Geometry: final body of the model. Coordinates: model frame, mm. Round coordinates to 2 decimals unless told otherwise and drop trailing zeros. Loops run counter-clockwise (first coordinate to the right, second up) from the corner with the lowest first, then second, coordinate; pieces in that order, holes last. Notation, with made-up numbers: (12, -37.75) - (25, -37.75) arc R14 cw to (25, -10.75) - close; hole circle Ø7 at (42.5, -25). An arc over 180 degrees is marked (long way). Answer in a Markdown table with one row per item. Add a question column.
from build123d import *

# Parameters (mm, degrees)
EXTRUDE_1_DEPTH     = 6.8
SKETCH_5_R          = 4
CUT_EXTRUDE_1_DEPTH = 13.03425666


with BuildPart() as part:
    # 草图1 → 凸台-拉伸1 (new body)
    with BuildSketch(Plane.XY):
        Polygon((0, 7.505553499), (-6.5, 3.75277675), (-6.5, -3.75277675), (0, -7.505553499), (6.5, -3.75277675), (6.5, 3.75277675), align=None)
    extrude(amount=EXTRUDE_1_DEPTH)

    # 草图4 → 切除-旋转1 (revolve, cut)
    with BuildSketch(Plane(origin=(0, 0, 0), x_dir=(0, 0, -1), z_dir=(1, 0, 0)), mode=Mode.PRIVATE) as cut_revolve_1_sk:
        Polygon((-6.8, -5.85), (-6.197427805, -7.505553499), (-6.8, -7.505553499), align=None)
    cut_revolve_1 = revolve(cut_revolve_1_sk.sketch.rotate(Axis((0, 0, 6.8), (0, 0, -1)), 119.999999984), axis=Axis((0, 0, 6.8), (0, 0, -1)), mode=Mode.SUBTRACT)

    # 镜向1: 切除-旋转1 across plane
    add(cut_revolve_1.mirror(Plane.XY.offset(3.4)), mode=Mode.SUBTRACT)

    # 草图5 → 切除-拉伸1 (cut, through all)
    with BuildSketch(Plane.XY.offset(6.8)):
        Circle(SKETCH_5_R)
    extrude(amount=-CUT_EXTRUDE_1_DEPTH, mode=Mode.SUBTRACT)


solid = part.part
1) Section B-B, the plane y = 0. Return the cut outline in (x, z).
2) Contact query for flat-ended pins moving along their axis: pin 1 Ø1.5 at (x, z) = (3, 2.5) entering from +Y; pin 2 Ø2 at (y, z) = (-5, 5) entering from +X; pin 3 Ø6.5 at (x, y) = (0, 0) entering from +Z. Output: stop coordinate, or through.
3) Pull-direction query (X, two-part tool) for faces 1 (the cylindrical face through (-0.867, -3.905, 3.448)), 2 (the flat face through (-3.2, 5.66, 3.36)), 3 (the flat face through (6.5, 0, 3)), 4 (the flat face through (3, -4, 6.8)); classes: pulls with the +X half, pulls with the -X half, needs draft (parallel to the pull), parting line crosses it, or undercut.
4) Material intervals for line 1 along Y through (x, z) = (1.75, 6); line 2 along X through (y, z) = (-1.25, 5.75); line 3 along Y through (x, z) = (-2.5, 2), sorted ascending. Write a range as from..to.
5) Section A-A, the plane z = 1.5. Return the cut outline in (x, y).
Evaluation:
| question | item | result |
|---|---|---|
| 1 | outline | (-6.5, 0.24) - (-5.85, 0) - (-4, 0) - (-4, 6.8) - (-5.85, 6.8) - (-6.5, 6.56) - close; (4, 0) - (5.85, 0) - (6.5, 0.24) - (6.5, 6.56) - (5.85, 6.8) - (4, 6.8) - close |
| 2 | pin 1 | stops at y = 6.21 |
| 2 | pin 2 | stops at x = 6.07 |
| 2 | pin 3 | passes through |
| 3 | face 1 | undercut |
| 3 | face 2 | pulls with the -X half |
| 3 | face 3 | pulls with the +X half |
| 3 | face 4 | needs draft |
| 4 | line 1 | y = -6.5..-3.6, 3.6..6.5 |
| 4 | line 2 | x = -6.5..-3.8, 3.8..6.5 |
| 4 | line 3 | y = -6.06..-3.12, 3.12..6.06 |
| 5 | outline | (-6.5, -3.75) - (0, -7.51) - (6.5, -3.75) - (6.5, 3.75) - (0, 7.51) - (-6.5, 3.75) - close; hole circle Ø8 at (0, 0) |
